```python
from build123d import *

# Parameters (mm, degrees)
EXTRUDE_1_DEPTH = 40
CHAMFER_1_SIZE  = 25
CHAMFER_2_SIZE  = 10
CHAMFER_3_SIZE  = 10


with BuildPart() as part:
    # 草图1 → 凸台-拉伸1 (new, symmetric)
    with BuildSketch(Plane.XY):
        with BuildLine():
            Line((-110, 50), (-110, 25))
            Line((-110, 25), (-65, 25))
            Line((-65, 25), (-65, -25))
            Line((-65, -25), (-110, -25))
            Line((-110, -25), (-110, -50))
            Line((-110, -50), (-9.158378918, -64.35156638))
            ThreePointArc((-9.158378918, -64.35156638), (65, 0), (-9.158378918, 64.35156638))
            Line((-9.158378918, 64.35156638), (-110, 50))
        make_face()
    extrude(amount=EXTRUDE_1_DEPTH, both=True)

    # 倒角1
    chamfer_1_edges = [part.edges().sort_by_distance(p)[0] for p in [
        (-110, 37.5, -40),
        (-110, -37.5, -40),
    ]]
    chamfer(chamfer_1_edges, length=CHAMFER_1_SIZE)

    # 倒角2
    chamfer_2_edges = [part.edges().sort_by_distance(p)[0] for p in [
        (-87.5, 25, 40),
        (-65, 0, 40),
        (-87.5, -25, 40),
    ]]
    chamfer(chamfer_2_edges, length=CHAMFER_2_SIZE)

    # 倒角3
    chamfer_3_edges = [part.edges().sort_by_distance(p)[0] for p in [
        (-75, 25, -40),
        (-75, -25, -40),
        (-65, 0, -40),
    ]]
    chamfer(chamfer_3_edges, length=CHAMFER_3_SIZE)


solid = part.part
```
CAD build for the part. Positions are in the model's coordinates, mm. A direction names the side the tool comes from. Coordinates: 2 decimals unless noted, no trailing zeros. Loops run counter-clockwise (first coordinate to the right, second up) from the corner with the lowest first, then second, coordinate; pieces in that order, holes last. Notation, with made-up numbers: (-25.75, 8) - (15.25, 8) arc R25 cw to (15.25, 23) - close; hole circle Ø3 at (65, 51). An arc over 180 degrees is marked (long way). Return JSON: item names as keys, results as strings.
1. Mould opens along Y. For faces 4 (the flat face through (-58.873, 57.276, 0.56)), 5 (the cylindrical face through (64.98, -1.56, 0.56)), 6 (the flat face through (-87, -25, 0)), 7 (the flat face through (-110, -37, 13)) say: released by +Y, released by -Y, zero draft, split by the parting line, or undercut.
Result:
{"face 4": "released by +Y", "face 5": "split by the parting line", "face 6": "undercut", "face 7": "zero draft"}
2. Band-saw the part on B-B (y = 0). Give the cut face in (x, z), and give its area (3 significant figures).
Result:
{"outline": "(-65, -30) - (-55, -40) - (65, -40) - (65, 40) - (-55, 40) - (-65, 30) - close", "area": "10,300 mm2"}
3. 3-axis set-ups, long thin cutter, end or side, ignore diameter. For faces 1 (the flat face through (-83, 30, 35)), 2 (the flat face through (-60, 0, -35)), 3 (the flat face through (-88, 25, 0)): which of +Z, -Z, +X, -X, +Y, -Y reach the whole face in a straight line?
Result:
{"face 1": "+Z, -X", "face 2": "-Z, -X", "face 3": "+Z, -Z, -X"}
4. Band-saw the part on D-D (z = -20). Give the cut face in (x, y), and give its area (3 significant figures).
Result:
{"outline": "(-105, -50.71) - (-9.16, -64.35) arc R65 ccw (long way) to (-9.16, 64.35) - (-105, 50.71) - (-105, 25) - (-65, 25) - (-65, -25) - (-105, -25) - close", "area": "16,900 mm2"}
5. Band-saw the part on A-A (z = 2). Give the cut face in (x, y), and give its area (3 significant figures).
Result:
{"outline": "(-110, -50) - (-9.16, -64.35) arc R65 ccw (long way) to (-9.16, 64.35) - (-110, 50) - (-110, 25) - (-65, 25) - (-65, -25) - (-110, -25) - close", "area": "17,100 mm2"}
6. Drop flat-ended pins along their axis: pin 1 (13.5 mm diameter, centred on x = -81.5, z = -11.5, fed in from -Y); pin 2 (5 mm diameter, centred on x = -56, y = 26.5, fed in from -Z); pin 3 (1 mm diameter, centred on x = 13.5, z = 27.5, fed in from -Y); pin 4 (1.5 mm diameter, centred on y = 49.5, z = -4, fed in from +X). Give the stop position or say it passes through.
Result:
{"pin 1": "stops at y = -55.02", "pin 2": "stops at z = -40", "pin 3": "stops at y = -63.69", "pin 4": "stops at x = 42.99"}
7. Probe L1, parallel to Y at x = 0.5, z = -21; L2, parallel to X at y = -2, z = 10; L3, parallel to Y at x = -66.5, z = -10. List the from-to ranges inside material, lowest first. Write a range as from..to.
Result:
{"L1": "y = -65..65", "L2": "x = -65..64.97", "L3": "y = -56.19..-25, 25..56.19"}
8. Band-saw the part on C-C (x = 47.5). Give the cut face in (y, z).
Result:
{"outline": "(-44.37, -40) - (44.37, -40) - (44.37, 40) - (-44.37, 40) - close"}
